Model file for the job. Use its own axes, mm. A direction names the side the tool comes from. Coordinates: 2 decimals unless noted, no trailing zeros. Write each loop counter-clockwise with the first axis right and the second up, starting at its lowest first coordinate (ties: lowest second). Pieces come first, ordered by that corner, then holes. Notation, with made-up numbers: (-3, 68) -> (32, 68) arc R21 ccw to (32, 102) -> close; hole circle Ø2 at (-34, 45). An arc over 180 degrees is marked (long way). Answer as a JSON object with one key per item and string values. Group by question number.
from build123d import *

# Parameters (mm, degrees)
EXTRUDE_1_DEPTH     = 360
CUT_EXTRUDE_1_DEPTH = 375.83329628


with BuildPart() as part:
    # 草图1 → 凸台-拉伸1 (new body)
    with BuildSketch(Plane.XY):
        with BuildLine():
            Line((5, 0), (95, 0))
            ThreePointArc((95, 0), (98.535533906, 1.464466094), (100, 5))
            Line((100, 5), (100, 30))
            Line((100, 30), (95, 30))
            Line((95, 30), (95, 10))
            ThreePointArc((95, 10), (93.535533906, 6.464466094), (90, 5))
            Line((90, 5), (10, 5))
            ThreePointArc((10, 5), (6.464466094, 6.464466094), (5, 10))
            Line((5, 10), (5, 30))
            Line((5, 30), (0, 30))
            Line((0, 30), (0, 5))
            ThreePointArc((0, 5), (1.464466094, 1.464466094), (5, 0))
        make_face()
    extrude(amount=EXTRUDE_1_DEPTH)

    # 草图2 → 切除-拉伸1 (cut, through all)
    with BuildSketch(Plane.ZY):
        Polygon((5, 5), (30, 30), (0, 30), (0, 5), align=None)
        Polygon((0, 0), (5, 5), (0, 5), align=None)
    extrude(amount=-CUT_EXTRUDE_1_DEPTH, mode=Mode.SUBTRACT)


solid = part.part
(1) Cut at B-B on z = 24.5. List the corners of the cut face in (x, y).
(2) Cut at C-C on x = 68. List the corners of the cut face in (y, z), plus the area to 3 significant figures.
(3) 3-axis set-ups, long thin cutter, end or side, ignore diameter. For faces 1 (the face through (95, 20, 183)), 2 (the face through (50, 4, 360)): which of +Z, -Z, +X, -X, +Y, -Y reach the whole face in a straight line?
(4) Pin check, flat tip, straight feed: pin 1 (3 mm diameter, centred on x = 82.5, z = 43.5, fed in from +Y). Stop position of the tip, or through.
(5) Cut at D-D on z = 186. List the corners of the cut face in (x, y).
(6) Cut at A-A on y = 18. List the corners of the cut face in (x, z).
(7) Wall check: probe 1 along X at (y, z) = (22, 331.5); probe 2 along Y at (x, z) = (75, 315); probe 3 along Z at (x, y) = (85, 4.5). Give the ranges that are in metal, low to high.
(8) Pull direction X, two halves, no side cores. Call faces 3 (the face through (100, 17, 180)), 4 (the face through (49, 0, 177)), 5 (the face through (5, 20, 183)): released by +X, released by -X, zero draft, split by the parting line, or undercut.
Results found:
{
 "1": {"outline": "(0, 5) arc R5 ccw to (5, 0) -> (95, 0) arc R5 ccw to (100, 5) -> (100, 24.5) -> (95, 24.5) -> (95, 10) arc R5 cw to (90, 5) -> (10, 5) arc R5 cw to (5, 10) -> (5, 24.5) -> (0, 24.5) -> close"},
 "2": {"outline": "(0, 0) -> (5, 5) -> (5, 360) -> (0, 360) -> close", "area": "1,790 mm²"},
 "3": {"face 1": "+Z, -Z, +Y", "face 2": "+Z, +X, -X, +Y, -Y"},
 "4": {"pin 1": "stops at y = 5"},
 "5": {"outline": "(0, 5) arc R5 ccw to (5, 0) -> (95, 0) arc R5 ccw to (100, 5) -> (100, 30) -> (95, 30) -> (95, 10) arc R5 cw to (90, 5) -> (10, 5) arc R5 cw to (5, 10) -> (5, 30) -> (0, 30) -> close"},
 "6": {"outline": "(0, 18) -> (5, 18) -> (5, 360) -> (0, 360) -> close; (95, 18) -> (100, 18) -> (100, 360) -> (95, 360) -> close"},
 "7": {"probe 1": "x = 0 to 5, 95 to 100", "probe 2": "y = 0 to 5", "probe 3": "z = 4.5 to 360"},
 "8": {"face 3": "released by +X", "face 4": "zero draft", "face 5": "undercut"}
}
